```python
from build123d import *

# Parameters (mm, degrees)
SKETCH2_R          = 20
CUT_EXTRUDE1_DEPTH = 662.64794264


with BuildPart() as part:
    # Sketch1 → Revolve1 (revolve)
    with BuildSketch(Plane.XY, mode=Mode.PRIVATE) as revolve1_sk:
        Polygon((0, 0), (25, 0), (25, 330), (33, 330), (33, 340), (25, 340), (25, 585.119663834), (25, 619.032357738), (25, 660), (0, 660), align=None)
    revolve(revolve1_sk.sketch.rotate(Axis((0, 660, 0), (0, -1, 0)), 180), axis=Axis((0, 660, 0), (0, -1, 0)))

    # Sketch2 → Cut-Extrude1 (cut, through all)
    with BuildSketch(Plane(origin=(0, 660, 0), x_dir=(1, 0, 0), z_dir=(0, 1, 0))):
        with Locations(Location((0, 0, 0), (0, 0, 180))):
            Circle(SKETCH2_R)
    extrude(amount=-CUT_EXTRUDE1_DEPTH, mode=Mode.SUBTRACT)


solid = part.part
```
For this review, take the finished solid that the model builds, in its own axes (mm). A direction names the side the tool comes from. Coordinates: 2 decimals unless noted, no trailing zeros. Loops run counter-clockwise (first coordinate to the right, second up) from the corner with the lowest first, then second, coordinate; pieces in that order, holes last. Notation, with made-up numbers: (9.5, 70.25) - (50.5, 70.25) arc R18 cw to (50.5, 90.25) - close; hole circle Ø9 at (8, 37.25). An arc over 180 degrees is marked (long way). Use one line per item in the form item = value. Start each with the question number.
1) For pin 1 (20 mm diameter, centred on x = 7, z = 15, fed in from -Y); pin 2 (10 mm diameter, centred on y = 304.5, z = 23, fed in from +X); pin 3 (1.5 mm diameter, centred on x = 25.5, z = 16, fed in from -Y); pin 4 (12 mm diameter, centred on y = 490, z = 9, fed in from -X), all flat-tipped, find the tip position at first contact; note any pin that passes through.
2) Take a section at B-B (x = 0). State the section outline as (y, z) points, plus the area to 3 significant figures.
3) Draft analysis for pull direction X (two halves, no side actions). For faces 4 (the face through (19.98, 334.62, 0.88)), 5 (the face through (-11, 0, -17)), 6 (the face through (-23.846, 502.24, -7.509)), state which applies: released by +X, released by -X, zero draft, split by the parting line, or undercut.
4) Take a section at C-C (y = 151). State the section outline as (x, z) points.
5) Take a section at A-A (z = 0). State the section outline as (x, y) points, plus the area to 3 significant figures.
6) For faces 1 (the face through (-5, 330, -25)), 2 (the face through (-31.476, 335.07, -9.912)), 3 (the face through (5, 340, -25)), list the 3-axis set-ups (+Z, -Z, +X, -X, +Y, -Y) from which the entire face can be reached by the end or side of a thin tool; tool diameter is ignored.
7) To check wall thickness, follow probe 1 along Z at (x, y) = (0, 393.5); probe 2 along Y at (x, z) = (27, -0.5); probe 3 along Z at (x, y) = (-14.5, 381). State the ranges of each line that lie inside material, in increasing order. Write a range as from..to.
From the geometry:
q1.pin_1 = 0
q1.pin_2 = 17.35
q1.pin_3 = 330
q1.pin_4 = -24.82
q2.outline = (0, -25) - (330, -25) - (330, -33) - (340, -33) - (340, -25) - (660, -25) - (660, -20) - (0, -20) - close; (0, 20) - (660, 20) - (660, 25) - (340, 25) - (340, 33) - (330, 33) - (330, 25) - (0, 25) - close
q2.area = 6,760 mm2
q3.face_4 = undercut
q3.face_5 = zero draft
q3.face_6 = split by the parting line
q4.outline = circle Ø50 at (0, 0); hole circle Ø40 at (0, 0)
q5.outline = (-33, 330) - (-25, 330) - (-25, 0) - (-20, 0) - (-20, 660) - (-25, 660) - (-25, 340) - (-33, 340) - close; (20, 0) - (25, 0) - (25, 330) - (33, 330) - (33, 340) - (25, 340) - (25, 660) - (20, 660) - close
q5.area = 6,760 mm2
q6.face_1 = -Y
q6.face_2 = +Y, -Y
q6.face_3 = +Y
q7.probe_1 = -25..-20, 20..25
q7.probe_2 = 330..340
q7.probe_3 = -20.37..-13.77, 13.77..20.37
